Geometry: see drawing. Coordinates: mm, zero at the bounding-box minimum. A direction names the side the tool comes from. Coordinates: 2 decimals unless noted, no trailing zeros. Write each loop counter-clockwise with the first axis right and the second up, starting at its lowest first coordinate (ties: lowest second). Pieces come first, ordered by that corner, then holes.
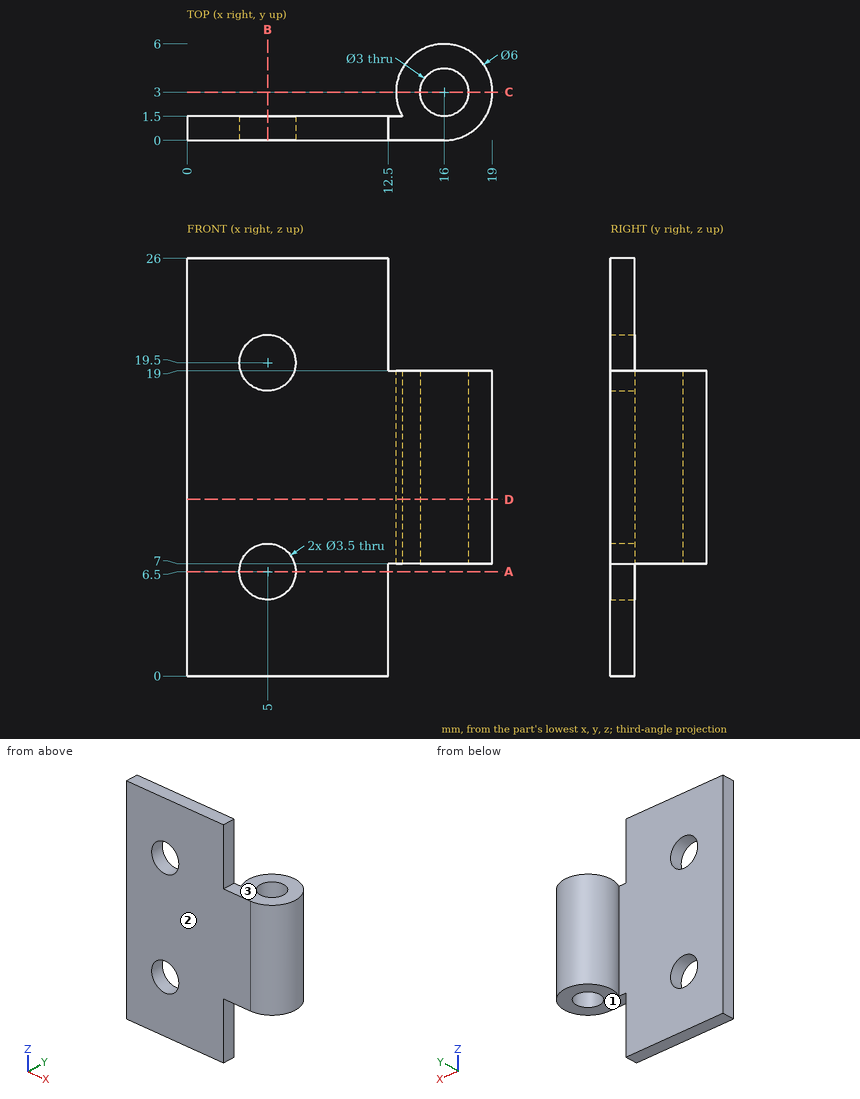
Item 1: Pin query (flat end, axial travel): pin 1 (4.5 mm diameter, centred on x = 5, z = 6.5, fed in from +Y); pin 2 (1.2 mm diameter, centred on y = 1, z = 23, fed in from +X); pin 3 (4 mm diameter, centred on x = 7, z = 12, fed in from -Y); pin 4 (3 mm diameter, centred on y = 1, z = 11.5, fed in from +X). Return the tip coordinate at first contact, or that it passes through.
Derived:
pin 1: stops at y = 1.5
pin 2: stops at x = 12.5
pin 3: stops at y = 0
pin 4: stops at x = 18.96
Item 2: Material intervals for probe 1 along Z at (x, y) = (5, 1); probe 2 along Z at (x, y) = (6.5, 0.9); probe 3 along Y at (x, z) = (4, 2), sorted ascending.
Derived:
probe 1: z = 0 to 4.75, 8.25 to 17.75, 21.25 to 26
probe 2: z = 0 to 5.6, 7.4 to 18.6, 20.4 to 26
probe 3: y = 0 to 1.5
Item 3: Section C-C, the plane y = 3. Output: boundary loops of the cut face in (x, z).
Derived:
outline: (13, 7) - (14.5, 7) - (14.5, 19) - (13, 19) - close; (17.5, 7) - (19, 7) - (19, 19) - (17.5, 19) - close
Item 4: Set-up query: the marked faces 1, 2 and 3. Return all of +Z, -Z, +X, -X, +Y, -Y with unobstructed straight access to the full face (end or side cutting, diameter ignored); none if empty.
Derived:
face 1: -Z, +X, +Y, -Y
face 2: +Z, -Z, +X, -X, -Y
face 3: +Z, +X, +Y, -Y
Item 5: Section A-A, the plane z = 6.5. Output: boundary loops of the cut face in (x, y), plus the area to 3 significant figures.
Derived:
outline: (0, 0) - (3.25, 0) - (3.25, 1.5) - (0, 1.5) - close; (6.75, 0) - (12.5, 0) - (12.5, 1.5) - (6.75, 1.5) - close
area: 13.5 mm2
Item 6: Section D-D, the plane z = 11. Output: boundary loops of the cut face in (x, y).
Derived:
outline: (0, 0) - (16, 0) arc R3 ccw (long way) to (13.4, 1.5) - (0, 1.5) - close; hole circle Ø3 at (16, 3)
Item 7: Section B-B, the plane x = 5. Output: boundary loops of the cut face in (y, z).
Derived:
outline: (0, 0) - (1.5, 0) - (1.5, 4.75) - (0, 4.75) - close; (0, 8.25) - (1.5, 8.25) - (1.5, 17.75) - (0, 17.75) - close; (0, 21.25) - (1.5, 21.25) - (1.5, 26) - (0, 26) - close
